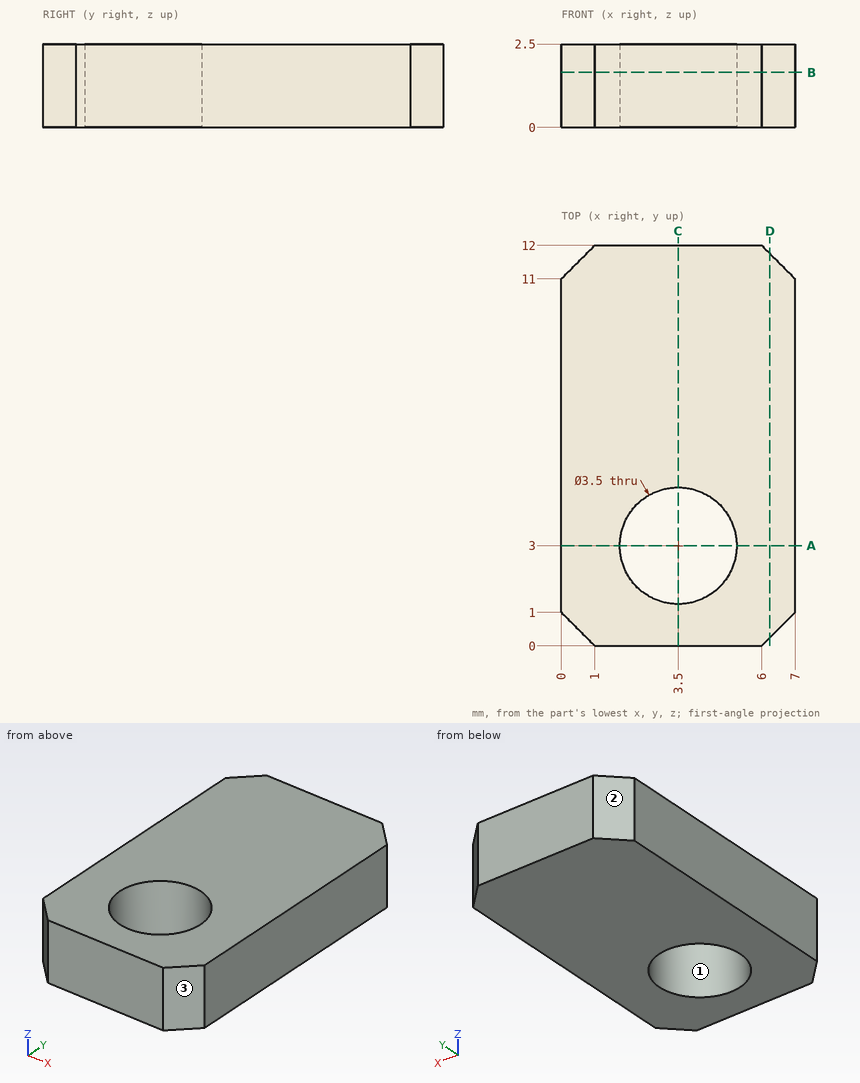
Source: three-view drawing plus pictorial views. Frame: mm from the lowest corner of the part. Coordinates: 2 decimals unless noted, no trailing zeros. Order: outer loops, then holes, each group sorted by start corner. A loop starts at its lowest first (then second) coordinate and runs counter-clockwise, first axis right, second up.
1) Section B-B (z = 1.65). Return loops of the section in (x, y), then the cut area to 3 significant figures.
Result sheet:
outline: (0, 1) - (1, 0) - (6, 0) - (7, 1) - (7, 11) - (6, 12) - (1, 12) - (0, 11) - close; hole circle Ø3.5 at (3.5, 3)
area: 72.4 mm2
2) Section A-A (y = 3). Return loops of the section in (x, z), then the cut area to 3 significant figures.
Result sheet:
outline: (0, 0) - (1.75, 0) - (1.75, 2.5) - (0, 2.5) - close; (5.25, 0) - (7, 0) - (7, 2.5) - (5.25, 2.5) - close
area: 8.75 mm2
3) Section D-D (x = 6.25). Return loops of the section in (y, z).
Result sheet:
outline: (0.25, 0) - (11.75, 0) - (11.75, 2.5) - (0.25, 2.5) - close
4) Draft query along X for the marked faces 1, 2 and 3. Return one class per face: released by +X, released by -X, zero draft, split by the parting line, or undercut.
Result sheet:
face 1: undercut
face 2: released by -X
face 3: released by +X
5) Section C-C (x = 3.5). Return loops of the section in (y, z), then the cut area to 4 significant figures.
Result sheet:
outline: (0, 0) - (1.25, 0) - (1.25, 2.5) - (0, 2.5) - close; (4.75, 0) - (12, 0) - (12, 2.5) - (4.75, 2.5) - close
area: 21.25 mm2
6) First-contact query: P1, Ø4, axis at x = 3.5, y = 3, coming from the +Z side. Flat tip, straight axial feed; report the tip coordinate or a pass-through.
Result sheet:
P1: stops at z = 2.5
7) Ray query, probe 1 along Y at (x, z) = (3.5, 1.5); probe 2 along Y at (x, z) = (5, 1.2); probe 3 along X at (y, z) = (2.5, 2.2). Return the intervals inside material, ascending.
Result sheet:
probe 1: y = 0 to 1.25, 4.75 to 12
probe 2: y = 0 to 2.1, 3.9 to 12
probe 3: x = 0 to 1.82, 5.18 to 7
